from build123d import *

# Parameters (mm, degrees)
SKETCH1_R           = 1.5
BOSS_EXTRUDE1_DEPTH = 50
SKETCH2_W           = 0.5
SKETCH2_H           = 4
CUT_EXTRUDE1_DEPTH  = 15
CHAMFER1_SIZE       = 0.2


with BuildPart() as part:
    # Sketch1 → Boss-Extrude1 (new body)
    with BuildSketch(Plane.XY):
        Circle(SKETCH1_R)
    extrude(amount=BOSS_EXTRUDE1_DEPTH)

    # Sketch2 → Cut-Extrude1 (cut, symmetric)
    with BuildSketch(Plane(origin=(0, 0, 0), x_dir=(1, 0, 0), z_dir=(0, 1, 0))):
        with Locations((-1.25, -4)):
            Rectangle(SKETCH2_W, SKETCH2_H)
    extrude(amount=CUT_EXTRUDE1_DEPTH, both=True, mode=Mode.SUBTRACT)

    # Chamfer1
    chamfer1_edges = [part.edges().sort_by_distance(p)[0] for p in [
        (-1.5, 0, 0),
        (-1.5, 0, 50),
    ]]
    chamfer(chamfer1_edges, length=CHAMFER1_SIZE)


solid = part.part
Could you check a few things on this model? Use its own coordinates, in mm. Give positions to 0.01 mm unless a question says otherwise; leave off trailing zeros. Loops run counter-clockwise (first coordinate to the right, second up) from the corner with the lowest first, then second, coordinate; pieces in that order, holes last. Notation, with made-up numbers: (61, 16) -> (120, 16) arc R16 cw to (120, 41) -> close; hole circle Ø8 at (72.5, -0.75). An arc over 180 degrees is marked (long way). Answer as CSV lines item,"result". Start each with the question number.
(1) I'm going to push flat-ended pins straight in: pin 1 Ø0.7 at (y, z) = (0, 5) entering from -X; pin 2 Ø1 at (x, z) = (1, 40) entering from +Y. Where does each tip first touch, or does it pass through?
(2) I need wall thicknesses on probe 1 along Z at (x, y) = (-1.15, 0.55); probe 2 along Y at (x, z) = (0.15, 33); probe 3 along Z at (x, y) = (-0.7, 1.1). Which ranges of each line are inside material? Lowest first, please.
(3) We'd pull the mould along Z, two halves only. Please class faces 1 (the flat face through (0, 0, 0)), 2 (the flat face through (-1, 0, 4)), 3 (the flat face through (0, 0, 50)), 4 (the cylindrical face through (1.43, 0.45, 24.65)): released by +Z, released by -Z, zero draft, split by the parting line, or undercut.
(4) If we section it at A-A on z = 35.5: Write out the boundary of the cut face in (x, y), then the cut area to 3 significant figures.
Computed:
1,pin 1,"stops at x = -1"
1,pin 2,"stops at y = 1.41"
2,probe 1,"z = 0 to 2, 6 to 50"
2,probe 2,"y = -1.49 to 1.49"
2,probe 3,"z = 0 to 50"
3,face 1,"released by -Z"
3,face 2,"undercut"
3,face 3,"released by +Z"
3,face 4,"zero draft"
4,outline,"circle Ø3 at (0, 0)"
4,area,"7.07 mm2"
